Verification items for the finished model (mm, model axes). A direction names the side the tool comes from. Round coordinates to 2 decimals unless told otherwise and drop trailing zeros. Write each loop counter-clockwise with the first axis right and the second up, starting at its lowest first coordinate (ties: lowest second). Pieces come first, ordered by that corner, then holes. Notation, with made-up numbers: M 48.25,10 L 78.25,10 A16 cw 78.25,35 Z; hole C -9,-28.5 d7. An arc over 180 degrees is marked long. Write each question's results on one line, items separated by ' | '.
from build123d import *

# Parameters (mm, degrees)
CUT_EXTRUDE1_START = -8.5
CUT_EXTRUDE1_DEPTH = 8.5


with BuildPart() as part:
    # Sketch1 → Revolve1 (revolve)
    with BuildSketch(Plane.XY, mode=Mode.PRIVATE) as revolve1_sk:
        with BuildLine():
            Line((0, 0), (0, 3))
            Line((0, 3), (10.5, 3))
            Line((10.5, 3), (10.5, 1.5))
            Line((10.5, 1.5), (13, 1.5))
            Line((13, 1.5), (13, 3))
            Line((13, 3), (15, 3))
            Line((15, 3), (15, 1.5))
            Line((15, 1.5), (27.5, 1.5))
            Line((27.5, 1.5), (27.5, 3))
            Line((27.5, 3), (29.5, 3))
            Line((29.5, 3), (29.5, 1.5))
            Line((29.5, 1.5), (34, 1.5))
            Line((34, 1.5), (34, 3))
            Line((34, 3), (36, 3))
            Line((36, 3), (36, 1.5))
            Line((36, 1.5), (38.5, 1.5))
            Line((38.5, 1.5), (38.5, 3))
            Line((38.5, 3), (39.5, 3))
            ThreePointArc((39.5, 3), (41.621320344, 2.121320344), (42.5, 0))
            Line((42.5, 0), (0, 0))
        make_face()
    revolve(revolve1_sk.sketch.rotate(Axis((0, 0, 0), (1, 0, 0)), 90), axis=Axis((0, 0, 0), (1, 0, 0)))

    # Sketch2 → Cut-Extrude1 (cut)
    with BuildSketch(Plane.ZY.offset(CUT_EXTRUDE1_START)):
        with BuildLine():
            Line((1, 2.828427125), (1, 1))
            Line((1, 1), (2.828427125, 1))
            ThreePointArc((2.828427125, 1), (2.121320344, 2.121320344), (1, 2.828427125))
        make_face()
        with BuildLine():
            Line((2.828427125, -1), (1, -1))
            Line((1, -1), (1, -2.828427125))
            ThreePointArc((1, -2.828427125), (2.121320344, -2.121320344), (2.828427125, -1))
        make_face()
        with BuildLine():
            ThreePointArc((-1, 2.828427125), (-2.121320344, 2.121320344), (-2.828427125, 1))
            Line((-2.828427125, 1), (-1, 1))
            Line((-1, 1), (-1, 2.828427125))
        make_face()
        with BuildLine():
            Line((-1, -1), (-2.828427125, -1))
            ThreePointArc((-2.828427125, -1), (-2.121320344, -2.121320344), (-1, -2.828427125))
            Line((-1, -2.828427125), (-1, -1))
        make_face()
    extrude(amount=CUT_EXTRUDE1_DEPTH, mode=Mode.SUBTRACT)


solid = part.part
1) Depth check by flat-ended pin: P1, Ø1.5, axis at x = 4, z = 2, coming from the -Y side; P2, Ø0.9, axis at x = 3.5, z = 2, coming from the +Y side; P3, Ø0.9, axis at y = -2.5, z = 2.5, coming from the -X side; P4, Ø0.9, axis at x = 3.5, y = 1.5, coming from the +Z side. Enter the tip coordinate at first touch or a pass-through.
Calculated:
P1: stops at y = -1 | P2: stops at y = 1 | P3: passes through | P4: stops at z = 1
2) Material ranges on line 1 (X direction, y = 0.55, z = 1.5); line 2 (X direction, y = -0.6, z = 2.1); line 3 (Y direction, x = 7, z = -2.1), recorded low to high. Write a range as [from, to].
Calculated:
line 1: x = [0, 10.5], [13, 15], [27.5, 29.5], [34, 36], [38.5, 42.04] | line 2: x = [0, 10.5], [13, 15], [27.5, 29.5], [34, 36], [38.5, 41.56] | line 3: y = [-1, 1]
3) Sectioned sample at A-A, the plane z = 2.3. Record the cut outline in (x, y).
Calculated:
outline: M 0,-1 L 8.5,-1 L 8.5,-1.93 L 10.5,-1.93 L 10.5,1.93 L 8.5,1.93 L 8.5,1 L 0,1 Z; M 13,-1.93 L 15,-1.93 L 15,1.93 L 13,1.93 Z; M 27.5,-1.93 L 29.5,-1.93 L 29.5,1.93 L 27.5,1.93 Z; M 34,-1.93 L 36,-1.93 L 36,1.93 L 34,1.93 Z; M 38.5,-1.93 L 39.5,-1.93 A1.93 ccw 39.5,1.93 L 38.5,1.93 Z
4) Sectioned sample at C-C, the plane x = 31. Record the cut outline in (y, z), and give its area (3 significant figures).
Calculated:
outline: C 0,0 d3 | area: 7.07 mm²
5) Draft check along X on faces 6 (the flat face through (8.5, -2, 2)), 7 (the flat face through (29.5, 1.3, 1.3)), 8 (the flat face through (4, -1, 2)). Enter one of: pulls with the +X half, pulls with the -X half, needs draft (parallel to the pull), parting line crosses it, or undercut.
Calculated:
face 6: pulls with the -X half | face 7: undercut | face 8: needs draft
6) Access from +Z, -Z, +X, -X, +Y, -Y to the whole of each face (thin tool, end or side, straight path). Record for faces 1 (the flat face through (4, -1, -2)), 2 (the cylindrical face through (39.01, -0.9, 2.86)), 3 (the flat face through (4, 2, 1)), 4 (the flat face through (4, 1, -2)), 5 (the flat face through (27.5, 1.3, -1.3)).
Calculated:
face 1: -Z, -X, -Y | face 2: +X, -X | face 3: +Z, -X, +Y | face 4: -Z, -X, +Y | face 5: none
